The listing builds one solid part. Answer for the finished solid, in the listing's coordinates (mm). Face numbers are marked on the shaded views. Round coordinates to 2 decimals unless told otherwise and drop trailing zeros. Order: outer loops, then holes, each group sorted by start corner. A loop starts at its lowest first (then second) coordinate and runs counter-clockwise, first axis right, second up. Notation, with made-up numbers: (20.25, 72.5) - (28.25, 72.5) arc R35 ccw to (28.25, 107.5) - close; hole circle Ø6 at (29, -34). An arc over 180 degrees is marked (long way). One line per item, written item: value. Start each with the question number.
1. For a pull along X with two mould halves and no side action, classify the marked faces 1 and 2 as released by +X, released by -X, zero draft, split by the parting line, or undercut.
2. Straight lines are drawn through the part: line 1 (X direction, y = 18.25, z = 0.05); line 2 (X direction, y = 4, z = -2.4); line 3 (Y direction, x = 1.3, z = 1.6). For each, find the intervals that lie inside material, in ascending order.
3. Section A-A, the plane x = 0 is taken. Give the vertices of the cut face in (y, z).
4. Flat-ended cylindrical pins translate along their axes: P1, Ø3, axis at y = 22.5, z = 1, coming from the +X side; P2, Ø1.5, axis at x = 2, y = 20, coming from the +Z side. Find the tip coordinate at first contact, or state that the pin passes through.
5. Section B-B, the plane z = 0 is taken. Give the vertices of the cut face in (x, y).
6. Section C-C, the plane y = 3 is taken. Give the vertices of the cut face in (x, z), then the cut area to 3 significant figures.
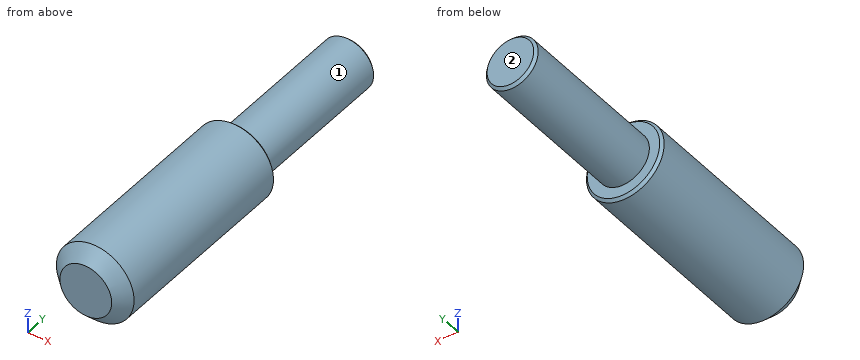
from build123d import *


with BuildPart() as part:
    # Sketch1 → Revolve1 (revolve)
    with BuildSketch(Plane.XY, mode=Mode.PRIVATE) as revolve1_sk:
        Polygon((0, 0), (-2, 0), (-3, 1), (-3, 15.8), (-2.8, 16), (-2, 16), (-2, 27.8), (-1.8, 28), (0, 28), align=None)
    revolve(revolve1_sk.sketch.rotate(Axis((0, 13.359319257, 0), (0, -1, 0)), 270), axis=Axis((0, 13.359319257, 0), (0, -1, 0)))


solid = part.part
Answer list:
1. face 1: split by the parting line
1. face 2: zero draft
2. line 1: x = -2 to 2
2. line 2: x = -1.8 to 1.8
2. line 3: y = 0.06 to 16
3. outline: (0, -2) - (1, -3) - (15.8, -3) - (16, -2.8) - (16, -2) - (27.8, -2) - (28, -1.8) - (28, 1.8) - (27.8, 2) - (16, 2) - (16, 2.8) - (15.8, 3) - (1, 3) - (0, 2) - close
4. P1: stops at x = 2
4. P2: stops at z = 1.56
5. outline: (-3, 1) - (-2, 0) - (2, 0) - (3, 1) - (3, 15.8) - (2.8, 16) - (2, 16) - (2, 27.8) - (1.8, 28) - (-1.8, 28) - (-2, 27.8) - (-2, 16) - (-2.8, 16) - (-3, 15.8) - close
6. outline: circle Ø6 at (0, 0)
6. area: 28.3 mm²
